Geometry: final body of the model. Coordinates: model frame, mm. Give positions to 0.01 mm unless a question says otherwise; leave off trailing zeros. Write each loop counter-clockwise with the first axis right and the second up, starting at its lowest first coordinate (ties: lowest second). Pieces come first, ordered by that corner, then holes. Notation, with made-up numbers: (57, -30.5) -> (84, -30.5) arc R20 cw to (84, 8.5) -> close; hole circle Ø6 at (17.25, 2). An arc over 180 degrees is marked (long way). Use CSV: the item, a comma, the result in double quotes. Start each with the question number.
1) Section D-D (z = -3). Output: boundary loops of the cut face in (x, y) (3 decimals), plus the area to 3 significant figures.
2) Contact query for flat-ended pins moving along their axis: P1, Ø8, axis at x = -16.5, y = -9.52, coming from the +Z side; P2, Ø3, axis at x = 15, z = -4.5, coming from the -Y side; P3, Ø1.5, axis at x = -6.5, z = -2.5, coming from the -Y side; P4, Ø1.5, axis at y = 5, z = -2.5, coming from the +X side. Output: stop coordinate, or through.
3) Draft query along X for faces 1 (the face through (-5.506, -24.796, -3.131)), 2 (the face through (-14.116, -10.512, -3.131)), 3 (the face through (5.3, -5.3, 0)). Return one class per face: pulls with the +X half, pulls with the -X half, needs draft (parallel to the pull), parting line crosses it, or undercut.
4) Material intervals for line 1 (Y direction, x = 0, z = -4.25); line 2 (X direction, y = -10, z = -5.75); line 3 (Y direction, x = -17, z = -5.5), sorted ascending. Write a range as [from, to].
5) Section B-B (x = 0). Output: boundary loops of the cut face in (y, z).
6) Section A-A (y = 0). Output: boundary loops of the cut face in (x, z), plus the area to 3 significant figures.
7) Section C-C (x = 15). Output: boundary loops of the cut face in (y, z).
```python
from build123d import *

# Parameters (mm, degrees)
SKETCH1_R           = 25.4
SKETCH1_R_2         = 7.1501
BOSS_EXTRUDE1_DEPTH = 6.35
SKETCH2_R           = 2.5781
CUT_EXTRUDE1_DEPTH  = 6.35


with BuildPart() as part:
    # Sketch1 → Boss-Extrude1 (new body)
    with BuildSketch(Plane.XY):
        Circle(SKETCH1_R)
        Circle(SKETCH1_R_2, mode=Mode.SUBTRACT)
    extrude(amount=-BOSS_EXTRUDE1_DEPTH)

    # Sketch2 → Cut-Extrude1 (cut)
    with BuildSketch(Plane.XY):
        with Locations((0, 19.05)):
            Circle(SKETCH2_R)
        with Locations((16.497783942, -9.525)):
            Circle(SKETCH2_R)
        with Locations((-16.497783942, -9.525)):
            Circle(SKETCH2_R)
    extrude(amount=-CUT_EXTRUDE1_DEPTH, mode=Mode.SUBTRACT)


solid = part.part
```
Answers follow:
1,outline,"circle Ø50.8 at (0, 0); hole circle Ø5.156 at (-16.498, -9.525); hole circle Ø14.3 at (0, 0); hole circle Ø5.156 at (0, 19.05); hole circle Ø5.156 at (16.498, -9.525)"
1,area,"1,800 mm^2"
2,P1,"stops at z = 0"
2,P2,"stops at y = -21.52"
2,P3,"stops at y = -24.74"
2,P4,"stops at x = 25.04"
3,face 1,"parting line crosses it"
3,face 2,"undercut"
3,face 3,"needs draft"
4,line 1,"y = [-25.4, -7.15], [7.15, 16.47], [21.63, 25.4]"
4,line 2,"x = [-23.35, -19.03], [-13.96, 13.96], [19.03, 23.35]"
4,line 3,"y = [-18.87, -12.05], [-7, 18.87]"
5,outline,"(-25.4, -6.35) -> (-7.15, -6.35) -> (-7.15, 0) -> (-25.4, 0) -> close; (7.15, -6.35) -> (16.47, -6.35) -> (16.47, 0) -> (7.15, 0) -> close; (21.63, -6.35) -> (25.4, -6.35) -> (25.4, 0) -> (21.63, 0) -> close"
6,outline,"(-25.4, -6.35) -> (-7.15, -6.35) -> (-7.15, 0) -> (-25.4, 0) -> close; (7.15, -6.35) -> (25.4, -6.35) -> (25.4, 0) -> (7.15, 0) -> close"
6,area,"232 mm^2"
7,outline,"(-20.5, -6.35) -> (-11.62, -6.35) -> (-11.62, 0) -> (-20.5, 0) -> close; (-7.43, -6.35) -> (20.5, -6.35) -> (20.5, 0) -> (-7.43, 0) -> close"
